The listing builds one solid part. Answer for the finished solid, in the listing's coordinates (mm). A direction names the side the tool comes from. Give positions to 0.01 mm unless a question says otherwise; leave off trailing zeros. Order: outer loops, then holes, each group sorted by start corner. A loop starts at its lowest first (then second) coordinate and runs counter-clockwise, first axis right, second up.
```python
from build123d import *

# Parameters (mm, degrees)
SKETCH_1_W                = 100
SKETCH_1_H                = 60
EXTRUDE_1_DEPTH           = 10
SKETCH_2_W                = 100
SKETCH_2_H                = 6.8
EXTRUDE_2_DEPTH           = 20
CHAMFER_1_SIZE            = 3
HOLE_WIZARD_M4_1_D        = 3.3
HOLE_WIZARD_M4_1_DEPTH    = 10.1
HOLE_WIZARD_M4_1_TIP      = 0.991420021
HOLE_WIZARD_1_D           = 5.5
HOLE_WIZARD_1_DEPTH       = 10.1
HOLE_WIZARD_1_CSINK_D     = 11.2
HOLE_WIZARD_1_CSINK_ANGLE = 90
HOLE_WIZARD_1_TIP         = 1.652366702


with BuildPart() as part:
    # 草图1 → 凸台-拉伸1 (new body)
    with BuildSketch(Plane(origin=(0, 0, 0), x_dir=(1, 0, 0), z_dir=(0, 1, 0))):
        Rectangle(SKETCH_1_W, SKETCH_1_H)
    extrude(amount=EXTRUDE_1_DEPTH)

    # 草图2 → 凸台-拉伸2 (add)
    with BuildSketch(Plane.XZ):
        with Locations((0, -26.6)):
            Rectangle(SKETCH_2_W, SKETCH_2_H)
    extrude(amount=EXTRUDE_2_DEPTH)

    # 倒角1
    chamfer_1_edges = [part.edges().sort_by_distance(p)[0] for p in [
        (50, -20, -26.6),
        (-50, -20, -26.6),
        (50, 5, 30),
        (-50, 5, 30),
    ]]
    chamfer(chamfer_1_edges, length=CHAMFER_1_SIZE)

    # M4 螺纹孔1
    with Locations(Plane(origin=(0, 10, 0), x_dir=(1, 0, 0), z_dir=(0, 1, 0))):
        with Locations((35, -2), (-37, -2), (-1, -2)):
            Hole(HOLE_WIZARD_M4_1_D / 2, depth=HOLE_WIZARD_M4_1_DEPTH)
            with Locations((0, 0, -(HOLE_WIZARD_M4_1_DEPTH + HOLE_WIZARD_M4_1_TIP / 2))):  # 118° drill point
                Cone(0, HOLE_WIZARD_M4_1_D / 2, HOLE_WIZARD_M4_1_TIP, mode=Mode.SUBTRACT)

    # 打孔尺寸(%根据)开槽半沉头木螺钉的类型1
    with Locations(Plane.XY.offset(-23.2)):
        with Locations((-10, -10), (-25, -10)):
            CounterSinkHole(HOLE_WIZARD_1_D / 2, HOLE_WIZARD_1_CSINK_D / 2, depth=HOLE_WIZARD_1_DEPTH, counter_sink_angle=HOLE_WIZARD_1_CSINK_ANGLE)
            with Locations((0, 0, -(HOLE_WIZARD_1_DEPTH + HOLE_WIZARD_1_TIP / 2))):  # 118° drill point
                Cone(0, HOLE_WIZARD_1_D / 2, HOLE_WIZARD_1_TIP, mode=Mode.SUBTRACT)


solid = part.part
```
1) Find section D-D (x = -43). Write down the section's boundary in (y, z).
Geometry says:
outline: (-20, -30) - (10, -30) - (10, 30) - (0, 30) - (0, -23.2) - (-20, -23.2) - close
2) Straight lines are drawn through the part: probe 1 along X at (y, z) = (-10, -28.9); probe 2 along Y at (x, z) = (-25, -28); probe 3 along Z at (x, y) = (-42, -9.75). For each, find the intervals that lie inside material, in ascending order.
Geometry says:
probe 1: x = -50 to -27.75, -22.25 to -12.75, -7.25 to 50
probe 2: y = -20 to -12.75, -7.25 to 10
probe 3: z = -30 to -23.2
3) For a pull along X with two mould halves and no side action, classify faces 1 (the cylindrical face through (-35.35, 4.93, 1.93)), 2 (the flat face through (50, 3, -8)), 3 (the flat face through (-1, -10, -23.2)) as +X half, -X half, draft (parallel to the pull), parting line (faces both ways), or undercut.
Geometry says:
face 1: undercut
face 2: +X half
face 3: draft
4) Given P1, Ø1, axis at x = 17.5, z = -9, coming from the -Y side; P2, Ø5, axis at x = 36.5, y = -10, coming from the +Z side, each flat-ended and moving along its own axis, determine where each tip first touches the part or whether it passes through.
Geometry says:
P1: stops at y = 0
P2: stops at z = -23.2
5) Find section A-A (x = -1). Write down the section's boundary in (y, z), then the cut area to 3 significant figures.
Geometry says:
outline: (-20, -30) - (10, -30) - (10, 0.35) - (0, 0.35) - (0, -23.2) - (-20, -23.2) - close; (0, 3.65) - (10, 3.65) - (10, 30) - (0, 30) - close
area: 703 mm2
6) A tool of negligible diameter and unlimited length cuts with its end or side. For faces 4 (the flat face through (-1, 0, -3)), 5 (the flat face through (-1, 10, 0)), from which of +Z, -Z, +X, -X, +Y, -Y can it reach the whole face along a straight path? Write none if from no direction.
Geometry says:
face 4: +Z, +X, -X, -Y
face 5: +Z, -Z, +X, -X, +Y
7) Find section B-B (z = 2). Write down the section's boundary in (x, y).
Geometry says:
outline: (-50, 0) - (-38.65, 0) - (-38.65, 10) - (-50, 10) - close; (-35.35, 0) - (-2.65, 0) - (-2.65, 10) - (-35.35, 10) - close; (0.65, 0) - (33.35, 0) - (33.35, 10) - (0.65, 10) - close; (36.65, 0) - (50, 0) - (50, 10) - (36.65, 10) - close
8) Find section C-C (x = -25). Write down the section's boundary in (y, z), then the cut area to 3 significant figures.
Geometry says:
outline: (-20, -30) - (-12.75, -30) - (-12.75, -26.05) - (-15.6, -23.2) - (-20, -23.2) - close; (-7.25, -30) - (10, -30) - (10, 30) - (0, 30) - (0, -23.2) - (-4.4, -23.2) - (-7.25, -26.05) - close
area: 690 mm2
